Work out the finished part from the listing and answer in its coordinate system (mm). A direction names the side the tool comes from. Round coordinates to 2 decimals unless told otherwise and drop trailing zeros. Order: outer loops, then holes, each group sorted by start corner. A loop starts at its lowest first (then second) coordinate and runs counter-clockwise, first axis right, second up. Notation, with made-up numbers: (17.5, 68.25) - (71.5, 68.25) arc R13 cw to (71.5, 80.25) - close; hole circle Ø7 at (-20, 36). An arc over 180 degrees is marked (long way). Use CSV: the item, a comma, the result in double quotes.
from build123d import *

# Parameters (mm, degrees)
BLOCK_PROFILE_SKETCH_70X65_W = 70
BLOCK_PROFILE_SKETCH_70X65_H = 65
BASE_BLOCK_70X65X80_DEPTH    = 40
UPPER_STEP_SKETCH_W          = 70
UPPER_STEP_SKETCH_H          = 30
UPPER_STEP_CUT_35_DEPTH      = 35
LOWER_STEP_CUT_20_DEPTH      = 20
ANGLED_CORNER_CUT_DEPTH      = 56


with BuildPart() as part:
    # Block Profile Sketch 70x65 → Base Block 70x65x80 (new, symmetric)
    with BuildSketch(Plane.XY):
        with Locations((35, 32.5)):
            Rectangle(BLOCK_PROFILE_SKETCH_70X65_W, BLOCK_PROFILE_SKETCH_70X65_H)
    extrude(amount=BASE_BLOCK_70X65X80_DEPTH, both=True)

    # Upper Step Sketch → Upper Step Cut 35 (cut)
    with BuildSketch(Plane.XY.offset(40)):
        with Locations((35, 50)):
            Rectangle(UPPER_STEP_SKETCH_W, UPPER_STEP_SKETCH_H)
    extrude(amount=-UPPER_STEP_CUT_35_DEPTH, mode=Mode.SUBTRACT)

    # Lower Step Sketch → Lower Step Cut 20 (cut)
    with BuildSketch(Plane.XY.offset(5)):
        Polygon((0, 35), (32, 65), (0, 65), align=None)
    extrude(amount=-LOWER_STEP_CUT_20_DEPTH, mode=Mode.SUBTRACT)

    # Corner Cut Sketch → Angled Corner Cut (cut)
    with BuildSketch(Plane(origin=(-13.333333333, 13.333333333, 13.333333333), x_dir=(-0.8164965809277261, -0.408248290463863, -0.408248290463863), z_dir=(0.5773502691896257, -0.5773502691896258, -0.5773502691896258))):
        Polygon((-16.329931619, 21.213203436), (-16.329931619, -28.284271247), (-59.196002117, -3.535533906), align=None)
    extrude(amount=-ANGLED_CORNER_CUT_DEPTH, mode=Mode.SUBTRACT)


solid = part.part
(1) Find section B-B (y = 34). Determine the outline of the cut face in (x, z).
Findings below:
outline,"(0, -40) - (70, -40) - (70, 40) - (34, 40) - (0, 6) - close"
(2) Find section C-C (x = 63.5). Determine the outline of the cut face in (y, z), and give its area (3 significant figures).
Findings below:
outline,"(0, -40) - (65, -40) - (65, 5) - (35, 5) - (35, 40) - (0, 40) - close"
area,"4,150 mm²"
(3) For faces 1 (the flat face through (42, 65, -22)), 2 (the flat face through (16, 50, -5)), 3 (the flat face through (42, 35, 23)), determine the directions among +Z, -Z, +X, -X, +Y, -Y from which every point of the face is accessible in a straight line to the end or side of a thin tool.
Findings below:
face 1,"+Z, -Z, +X, -X, +Y"
face 2,"+Z, -X, +Y"
face 3,"+Z, +X, -X, +Y"
(4) Each of these flat-tipped pins is pushed along its axis until it touches: pin 1 (1 mm diameter, centred on x = 62.5, y = 45, fed in from +Z); pin 2 (24 mm diameter, centred on x = 14, y = 43.5, fed in from +Z); pin 3 (1.5 mm diameter, centred on x = 24, z = -11.5, fed in from +Y). Where does it stop, or does it pass through?
Findings below:
pin 1,"stops at z = 5"
pin 2,"stops at z = 27.47"
pin 3,"stops at y = 58.2"
(5) Find section D-D (y = 57). Determine the outline of the cut face in (x, z), and give its area (3 significant figures).
Findings below:
outline,"(0, -40) - (70, -40) - (70, 5) - (23.47, 5) - (23.47, -15) - (0, -15) - close"
area,"2,680 mm²"
(6) Find section A-A (z = 20.5). Determine the outline of the cut face in (x, y).
Findings below:
outline,"(0, 0) - (70, 0) - (70, 35) - (15.5, 35) - (0, 19.5) - close"
(7) Find the intervals of material crossed by L1, parallel to Z at x = 28.5, y = 61; L2, parallel to Y at x = 39, z = 13; L3, parallel to Z at x = 18.5, y = 57, in increasing order. Write a range as from..to.
Findings below:
L1,"z = -40..5"
L2,"y = 0..35"
L3,"z = -40..-15"
